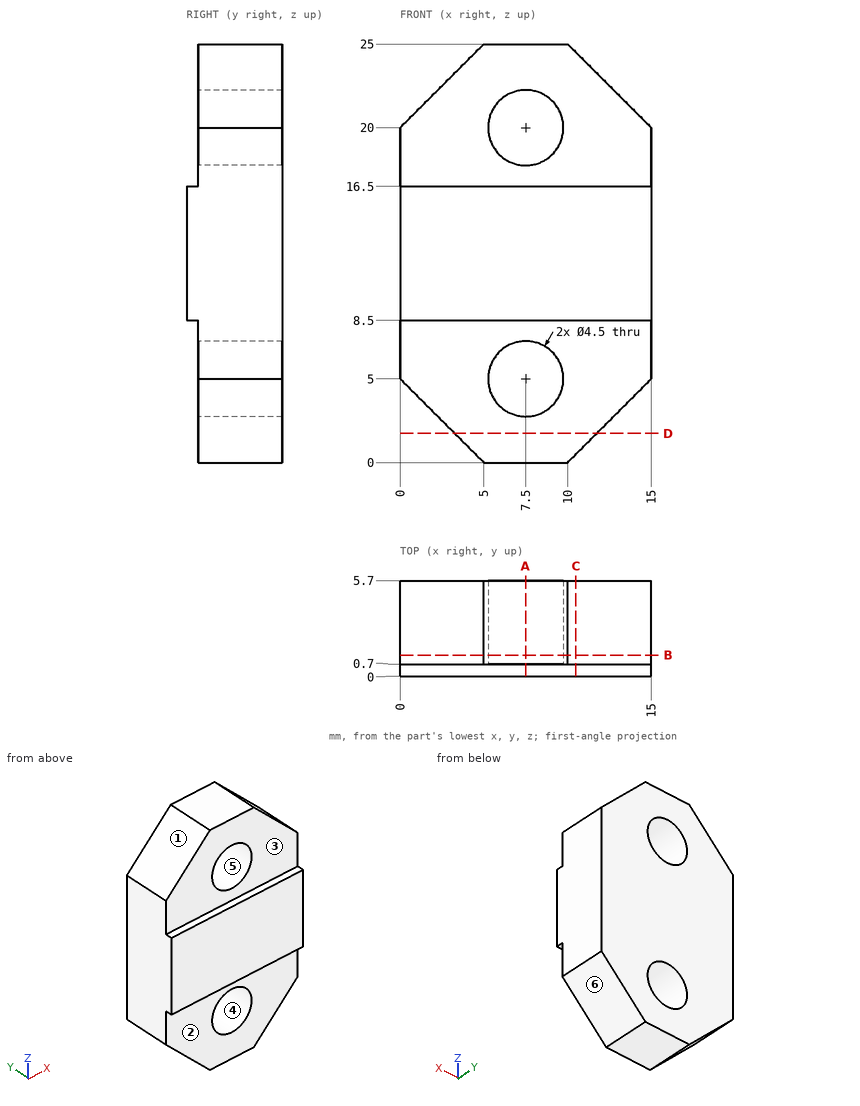
Verification items for this drawing (mm, ordinates from the low corner). A direction names the side the tool comes from. Coordinates: 2 decimals unless noted, no trailing zeros. Write each loop counter-clockwise with the first axis right and the second up, starting at its lowest first coordinate (ties: lowest second). Pieces come first, ordered by that corner, then holes. Notation, with made-up numbers: M 83,65.5 L 117,65.5 A25 ccw 117,96.5 Z; hole C 27.25,87 d2. An arc over 180 degrees is marked long. Use one line per item in the form item = value. Start each with the question number.
1) Section check C-C on x = 10.5. Enter the section's corners in (y, z).
2) Section check D-D on z = 1.75. Enter the section's corners in (x, y).
3) Section check A-A on x = 7.5. Enter the section's corners in (y, z), and give its area (3 significant figures).
4) Set-up check for the marked faces 1 and 2: record each of +Z, -Z, +X, -X, +Y, -Y from which the full face is reachable in a straight line by a thin tool's end or side.
5) Section check B-B on y = 1.25. Enter the section's corners in (x, z).
6) Thickness scan on probe 1 along Z at (x, y) = (7.5, 1.95); probe 2 along Z at (x, y) = (6, 1.75); probe 3 along Y at (x, z) = (12, 5.25). Record the ranges inside material, lowest first. Write a range as from..to.
7) Release check for a two-part mould opening along Z. For the marked faces 3, 4, 5 and 6 record: pulls with the +Z half, pulls with the -Z half, needs draft (parallel to the pull), parting line crosses it, or undercut.
8) Go/stop test with flat-tipped pins: pin 1 Ø2.5 at (x, z) = (5.5, 22) entering from -Y; pin 2 Ø3 at (x, y) = (12.5, 4) entering from -Z; pin 3 Ø4 at (x, z) = (7.5, 5) entering from -Y (1 decimal). Record where each tip stops, or that it passes through.
Responses:
q1.outline = M 0,8.5 L 0.7,8.5 L 0.7,0.5 L 5.7,0.5 L 5.7,24.5 L 0.7,24.5 L 0.7,16.5 L 0,16.5 Z
q2.outline = M 3.25,0.7 L 11.75,0.7 L 11.75,5.7 L 3.25,5.7 Z
q3.outline = M 0,8.5 L 0.7,8.5 L 0.7,7.25 L 5.7,7.25 L 5.7,17.75 L 0.7,17.75 L 0.7,16.5 L 0,16.5 Z; M 0.7,0 L 5.7,0 L 5.7,2.75 L 0.7,2.75 Z; M 0.7,22.25 L 5.7,22.25 L 5.7,25 L 0.7,25 Z
q3.area = 85.6 mm2
q4.face_1 = +Z, -X, +Y, -Y
q4.face_2 = -Z, +X, -X, -Y
q5.outline = M 0,5 L 5,0 L 10,0 L 15,5 L 15,20 L 10,25 L 5,25 L 0,20 Z; hole C 7.5,5 d4.5; hole C 7.5,20 d4.5
q6.probe_1 = 0..2.75, 7.25..17.75, 22.25..25
q6.probe_2 = 0..3.32, 6.68..18.32, 21.68..25
q6.probe_3 = 0.7..5.7
q7.face_3 = needs draft
q7.face_4 = undercut
q7.face_5 = undercut
q7.face_6 = pulls with the -Z half
q8.pin_1 = 0.7
q8.pin_2 = 1
q8.pin_3 = through
